Can you work these out from the model? Positions are in its coordinate system, mm. Face numbers are marked on the shaded views. A direction names the side the tool comes from. Give positions to 0.01 mm unless a question says otherwise; leave off trailing zeros. Order: outer loops, then holes, each group sorted by start corner. A loop starts at its lowest first (then second) coordinate and runs counter-clockwise, first axis right, second up. Notation, with made-up numbers: (49, -2.75) - (102, -2.75) arc R15 cw to (102, 23.25) - close; hole circle Ø5 at (32, 71.5). An arc over 180 degrees is marked (long way). Answer as a JSON object with one key per item and string values.
```python
from build123d import *

# Parameters (mm, degrees)
SKETCH1_R           = 115
SKETCH1_R_2         = 72
SKETCH1_R_3         = 7.25
BOSS_EXTRUDE1_DEPTH = 60
SKETCH2_R           = 11
CUT_EXTRUDE1_DEPTH  = 30


with BuildPart() as part:
    # Sketch1 → Boss-Extrude1 (new body)
    with BuildSketch(Plane(origin=(0, 0, 0), x_dir=(1, 0, 0), z_dir=(0, 1, 0))):
        with Locations(Location((0, 0, 0), (0, 0, 270))):
            Circle(SKETCH1_R)
        with Locations(Location((0, 0, 0), (0, 0, 270))):
            Circle(SKETCH1_R_2, mode=Mode.SUBTRACT)
        with Locations(Location((0, 88, 0), (0, 0, 270))):
            Circle(SKETCH1_R_3, mode=Mode.SUBTRACT)
        with Locations(Location((44, 76.210235533, 0), (0, 0, 270))):
            Circle(SKETCH1_R_3, mode=Mode.SUBTRACT)
        with Locations(Location((76.210235533, 44, 0), (0, 0, 270))):
            Circle(SKETCH1_R_3, mode=Mode.SUBTRACT)
        with Locations(Location((88, 0, 0), (0, 0, 270))):
            Circle(SKETCH1_R_3, mode=Mode.SUBTRACT)
        with Locations(Location((76.210235533, -44, 0), (0, 0, 270))):
            Circle(SKETCH1_R_3, mode=Mode.SUBTRACT)
        with Locations(Location((44, -76.210235533, 0), (0, 0, 270))):
            Circle(SKETCH1_R_3, mode=Mode.SUBTRACT)
        with Locations(Location((0, -88, 0), (0, 0, 270))):
            Circle(SKETCH1_R_3, mode=Mode.SUBTRACT)
        with Locations(Location((-44, -76.210235533, 0), (0, 0, 270))):
            Circle(SKETCH1_R_3, mode=Mode.SUBTRACT)
        with Locations(Location((-76.210235533, -44, 0), (0, 0, 270))):
            Circle(SKETCH1_R_3, mode=Mode.SUBTRACT)
        with Locations(Location((-88, 0, 0), (0, 0, 270))):
            Circle(SKETCH1_R_3, mode=Mode.SUBTRACT)
        with Locations(Location((-76.210235533, 44, 0), (0, 0, 270))):
            Circle(SKETCH1_R_3, mode=Mode.SUBTRACT)
        with Locations(Location((-44, 76.210235533, 0), (0, 0, 270))):
            Circle(SKETCH1_R_3, mode=Mode.SUBTRACT)
    extrude(amount=BOSS_EXTRUDE1_DEPTH)

    # Sketch2 → Cut-Extrude1 (cut)
    with BuildSketch(Plane.XZ):
        with Locations(Location((0, 88, 0), (0, 0, 270))):
            Circle(SKETCH2_R)
        with Locations(Location((44, 76.210235533, 0), (0, 0, 270))):
            Circle(SKETCH2_R)
        with Locations(Location((76.210235533, 44, 0), (0, 0, 270))):
            Circle(SKETCH2_R)
        with Locations(Location((88, 0, 0), (0, 0, 270))):
            Circle(SKETCH2_R)
        with Locations(Location((76.210235533, -44, 0), (0, 0, 270))):
            Circle(SKETCH2_R)
        with Locations(Location((44, -76.210235533, 0), (0, 0, 270))):
            Circle(SKETCH2_R)
        with Locations(Location((0, -88, 0), (0, 0, 270))):
            Circle(SKETCH2_R)
        with Locations(Location((-44, -76.210235533, 0), (0, 0, 270))):
            Circle(SKETCH2_R)
        with Locations(Location((-76.210235533, -44, 0), (0, 0, 270))):
            Circle(SKETCH2_R)
        with Locations(Location((-88, 0, 0), (0, 0, 270))):
            Circle(SKETCH2_R)
        with Locations(Location((-76.210235533, 44, 0), (0, 0, 270))):
            Circle(SKETCH2_R)
        with Locations(Location((-44, 76.210235533, 0), (0, 0, 270))):
            Circle(SKETCH2_R)
    extrude(amount=-CUT_EXTRUDE1_DEPTH, mode=Mode.SUBTRACT)


solid = part.part
```
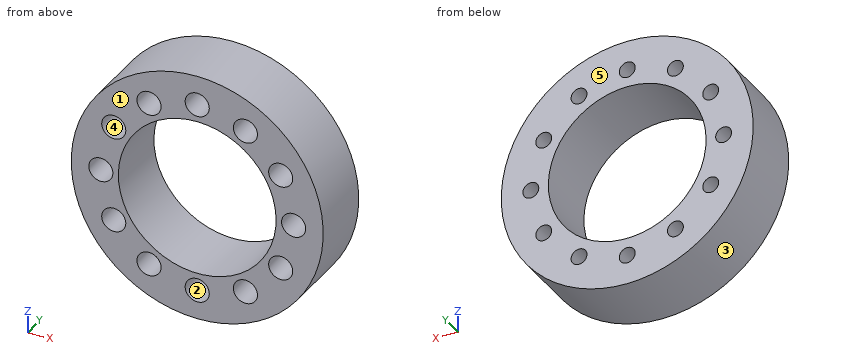
Q1. I'm going to push flat-ended pins straight in: pin 1 Ø2 at (y, z) = (36, -11) entering from +X; pin 2 Ø10 at (x, y) = (-44.5, 21) entering from -Z; pin 3 Ø6 at (y, z) = (14.5, 70.5) entering from +X. Where does each tip first touch, or does it pass through?
Recorded:
{"pin 1": "stops at x = 114.56", "pin 2": "stops at z = -108", "pin 3": "stops at x = 93.11"}
Q2. If we section it at A-A, the plane z = 0: Please give me the cut outline in (x, y).
Recorded:
{"outline": "(-115, 0) - (-99, 0) - (-99, 30) - (-95.25, 30) - (-95.25, 60) - (-115, 60) - close; (-80.75, 30) - (-77, 30) - (-77, 0) - (-72, 0) - (-72, 60) - (-80.75, 60) - close; (72, 0) - (77, 0) - (77, 30) - (80.75, 30) - (80.75, 60) - (72, 60) - close; (95.25, 30) - (99, 30) - (99, 0) - (115, 0) - (115, 60) - (95.25, 60) - close"}
Q3. If we section it at D-D, the plane y = 40.5: Count the separate pieces of the cut face and the enclosed holes in it, then the cut area to 3 significant figures.
Recorded:
{"separate pieces": "1", "enclosed holes": "13", "area": "23,300 mm^2"}
Q4. If we section it at C-C, the plane z = 24.5: Please give me the cut outline in (x, y), then the cut area to 3 significant figures.
Recorded:
{"outline": "(-112.36, 0) - (-67.7, 0) - (-67.7, 60) - (-112.36, 60) - close; (67.7, 0) - (112.36, 0) - (112.36, 60) - (67.7, 60) - close", "area": "5,360 mm^2"}
Q5. I need wall thicknesses on L1, parallel to Z at x = -0.5, y = 37; L2, parallel to Z at x = 43.5, y = 48; L3, parallel to X at y = 19, z = 40. Which ranges of each line are inside material? Lowest first, please.
Recorded:
{"L1": "z = -115 to -95.23, -80.77 to -72, 72 to 80.77, 95.23 to 115", "L2": "z = -106.46 to -83.44, -68.98 to -57.37, 57.37 to 68.98, 83.44 to 106.46", "L3": "x = -107.82 to -86.46, -65.96 to -59.87, 59.87 to 65.96, 86.46 to 107.82"}
Q6. If we section it at B-B, the plane x = -44: Please give me the cut outline in (y, z), then the cut area to 3 significant figures.
Recorded:
{"outline": "(0, -106.25) - (60, -106.25) - (60, -83.46) - (30, -83.46) - (30, -87.21) - (0, -87.21) - close; (0, -65.21) - (30, -65.21) - (30, -68.96) - (60, -68.96) - (60, -56.99) - (0, -56.99) - close; (0, 56.99) - (60, 56.99) - (60, 68.96) - (30, 68.96) - (30, 65.21) - (0, 65.21) - close; (0, 87.21) - (30, 87.21) - (30, 83.46) - (60, 83.46) - (60, 106.25) - (0, 106.25) - close", "area": "3,720 mm^2"}
Q7. We'd pull the mould along Z, two halves only. Please class the marked faces 1, 2 and 3: released by +Z, released by -Z, zero draft, split by the parting line, or undercut.
Recorded:
{"face 1": "zero draft", "face 2": "undercut", "face 3": "split by the parting line"}
Q8. Which directions (+Z, -Z, +X, -X, +Y, -Y) give clear straight access to the entire face, cutting with the end or side of a thin tool? Please do the marked faces 4 and 5.
Recorded:
{"face 4": "-Y", "face 5": "+Z, -Z, +X, -X, +Y"}
